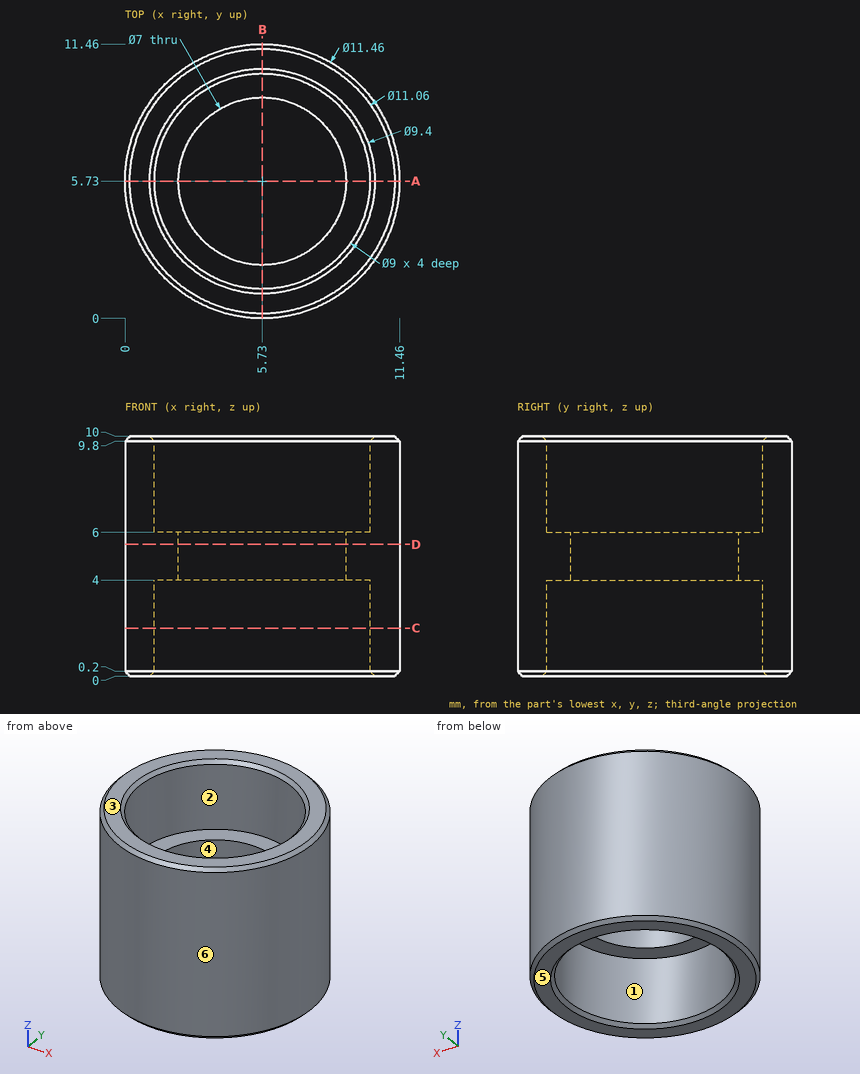
Source: three-view drawing plus pictorial views. Frame: mm from the lowest corner of the part. A direction names the side the tool comes from. Give positions to 0.01 mm unless a question says otherwise; leave off trailing zeros. Order: outer loops, then holes, each group sorted by start corner. A loop starts at its lowest first (then second) coordinate and runs counter-clockwise, first axis right, second up. Notation, with made-up numbers: M 60,61.25 L 88,61.25 A26 ccw 88,79.25 Z; hole C -11.75,46 d3. An arc over 180 degrees is marked long. Return JSON: item names as keys, results as strings.
1) Section query C-C on z = 2. Output: boundary loops of the cut face in (x, y), and give its area (3 significant figures).
Taken from the geometry:
{"outline": "C 5.73,5.73 d11.46; hole C 5.73,5.73 d9", "area": "39.5 mm2"}
2) Contact query for flat-ended pins moving along their axis: pin 1 (6 mm diameter, centred on x = 2, z = 6, fed in from +Y); pin 2 (4.5 mm diameter, centred on x = 6, y = 7.5, fed in from -Z); pin 3 (1 mm diameter, centred on x = 2, z = 7, fed in from -Y). Output: stop coordinate, or through.
Taken from the geometry:
{"pin 1": "stops at y = 11.41", "pin 2": "stops at z = 4", "pin 3": "stops at y = 1"}
3) Access query for the marked faces 1, 2 and 3. Directions: +Z, -Z, +X, -X, +Y, -Y. A direction counts if a zero-diameter tool reaches every point of the face in a straight line with its end or side. Return the directions, or none.
Taken from the geometry:
{"face 1": "-Z", "face 2": "+Z", "face 3": "+Z, +X, -X, +Y, -Y"}
4) Mould query, pull axis Y, two halves, no side actions, for the marked faces 4, 5 and 6. Classes: released by +Y, released by -Y, zero draft, split by the parting line, or undercut.
Taken from the geometry:
{"face 4": "undercut", "face 5": "zero draft", "face 6": "split by the parting line"}
5) Section query A-A on y = 5.73. Output: boundary loops of the cut face in (x, z).
Taken from the geometry:
{"outline": "M 0,0.2 L 0.2,0 L 1.03,0 L 1.23,0.2 L 1.23,4 L 2.23,4 L 2.23,6 L 1.23,6 L 1.23,9.8 L 1.03,10 L 0.2,10 L 0,9.8 Z; M 9.23,4 L 10.23,4 L 10.23,0.2 L 10.43,0 L 11.26,0 L 11.46,0.2 L 11.46,9.8 L 11.26,10 L 10.43,10 L 10.23,9.8 L 10.23,6 L 9.23,6 Z"}
6) Line query: L1, parallel to Y at x = 5.73, z = 9.05; L2, parallel to Y at x = 5, z = 3.25. Output: solid intervals per line, ascending. Write a range as [from, to].
Taken from the geometry:
{"L1": "y = [0, 1.23], [10.23, 11.46]", "L2": "y = [0.05, 1.29], [10.17, 11.41]"}
7) Section query D-D on z = 5.5. Output: boundary loops of the cut face in (x, y), and give its area (3 significant figures).
Taken from the geometry:
{"outline": "C 5.73,5.73 d11.46; hole C 5.73,5.73 d7", "area": "64.7 mm2"}
